Design review of the part built by this model. Coordinates are the model's own, in mm. A direction names the side the tool comes from. Round coordinates to 2 decimals unless told otherwise and drop trailing zeros. Loops run counter-clockwise (first coordinate to the right, second up) from the corner with the lowest first, then second, coordinate; pieces in that order, holes last. Notation, with made-up numbers: M 26.5,-13.5 L 69.5,-13.5 A11 cw 69.5,-0.5 Z; hole C 63.5,64 d7. An arc over 180 degrees is marked long. Use a Markdown table: item, result.
from build123d import *

# Parameters (mm, degrees)
SKETCH_1_W      = 50
SKETCH_1_H      = 50
SKETCH_1_W_2    = 44
SKETCH_1_H_2    = 44
EXTRUDE_1_DEPTH = 415


with BuildPart() as part:
    # 草图1 → 凸台-拉伸1 (new body)
    with BuildSketch(Plane.XY):
        with Locations((25, 25)):
            Rectangle(SKETCH_1_W, SKETCH_1_H)
        with Locations((25, 25)):
            Rectangle(SKETCH_1_W_2, SKETCH_1_H_2, mode=Mode.SUBTRACT)
    extrude(amount=EXTRUDE_1_DEPTH)


solid = part.part
1. Take a section at C-C on z = 361.5. Give the boundary of the cut face in (x, y), and give its area (3 significant figures).
Check values:
| item | result |
|---|---|
| outline | M 0,0 L 50,0 L 50,50 L 0,50 Z; hole M 3,3 L 47,3 L 47,47 L 3,47 Z |
| area | 564 mm² |
2. Take a section at A-A on y = 31.5. Give the boundary of the cut face in (x, z).
Check values:
| item | result |
|---|---|
| outline | M 0,0 L 3,0 L 3,415 L 0,415 Z; M 47,0 L 50,0 L 50,415 L 47,415 Z |
3. Machinability: for faces 1 (the face through (0, 25, 205)), 2 (the face through (3, 25, 205)), which of the approach directions +Z, -Z, +X, -X, +Y, -Y give a long, thin tool a straight path to every point of the face, cutting with its end or side? Answer none if there is none.
Check values:
| item | result |
|---|---|
| face 1 | +Z, -Z, -X, +Y, -Y |
| face 2 | +Z, -Z |
4. The part is to be moulded in two halves that separate along Y. For faces 3 (the face through (25, 0, 205)), 4 (the face through (2.7, 25.1, 415)), 5 (the face through (25, 47, 205)), say which applies: pulls with the +Y half, pulls with the -Y half, needs draft (parallel to the pull), parting line crosses it, or undercut.
Check values:
| item | result |
|---|---|
| face 3 | pulls with the -Y half |
| face 4 | needs draft |
| face 5 | undercut |
5. Wall thickness on line 1 along Y through (x, z) = (7, 141): over which ranges is the line inside the solid? List them lowest first. Write a range as from..to.
Check values:
| item | result |
|---|---|
| line 1 | y = 0..3, 47..50 |
